Here's the drawing with two shaded views (mm, measured from the low corner). I have some questions. Give positions to 0.01 mm unless a question says otherwise; leave off trailing zeros. Loops run counter-clockwise (first coordinate to the right, second up) from the corner with the lowest first, then second, coordinate; pieces in that order, holes last. Notation, with made-up numbers: M -38,31 L -13,31 A23 ccw -13,46 Z; hole C -31.75,9 d1. An arc over 180 degrees is marked long. Answer in a Markdown table with one row per item. Add a question column.
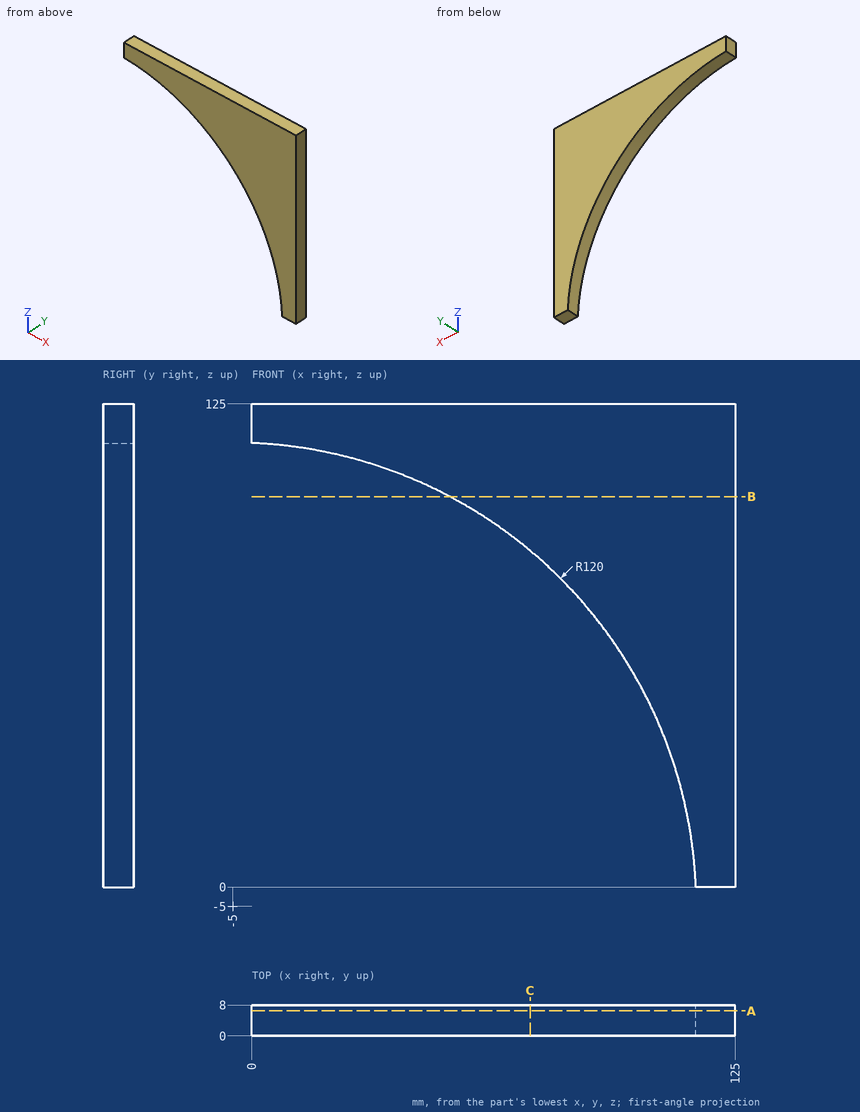
Item 1: I need wall thicknesses on L1, parallel to Z at x = 37.5, y = 0.5; L2, parallel to X at y = 6, z = 41; L3, parallel to Z at x = 43.5, y = 4.5. Which ranges of each line are inside material? Lowest first, please.
Item 2: Suppose I cut it at B-B (z = 101). List the corners of the cut face in (x, y) for me.
Item 3: Suppose I cut it at C-C (x = 72). List the corners of the cut face in (y, z) for me.
Item 4: Suppose I cut it at A-A (y = 6.5). List the corners of the cut face in (x, z) for me.
Values found:
| question | item | result |
|---|---|---|
| 1 | L1 | 107.22 to 125 |
| 1 | L2 | 105.83 to 125 |
| 1 | L3 | 104.76 to 125 |
| 2 | outline | M 51.25,0 L 125,0 L 125,8 L 51.25,8 Z |
| 3 | outline | M 0,87.04 L 8,87.04 L 8,125 L 0,125 Z |
| 4 | outline | M 0,114.9 A120 cw 114.9,0 L 125,0 L 125,125 L 0,125 Z |
